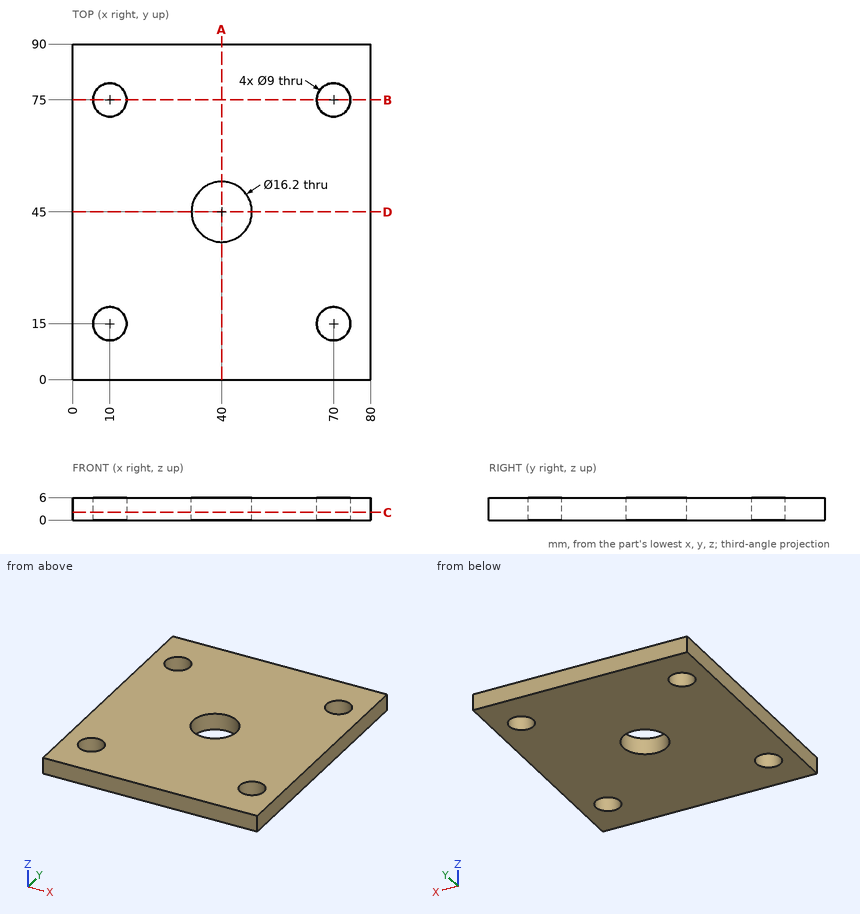
Part print with two shaded views. Sizes in mm from the minimum x, y, z corner. Round coordinates to 2 decimals unless told otherwise and drop trailing zeros. Order: outer loops, then holes, each group sorted by start corner. A loop starts at its lowest first (then second) coordinate and runs counter-clockwise, first axis right, second up. Notation, with made-up numbers: M 55,-1 L 60,-1 A27 ccw 60,15 Z; hole C 71.5,25.25 d5. An arc over 180 degrees is marked long. Use CSV: the item, a comma, the result in double quotes. Start each with the question number.
(1) Cut at D-D on y = 45. List the corners of the cut face in (x, z), then the cut area to 3 significant figures.
(2) Drill centre lines: probe 1 along X at (y, z) = (75, 3.9); probe 2 along Y at (x, z) = (8.5, 3.9); probe 3 along Y at (x, z) = (73.5, 3.6). Where is each one in solid material? Low to high.
(3) Cut at C-C on z = 2.05. List the corners of the cut face in (x, y), then the cut area to 3 significant figures.
(4) Cut at A-A on x = 40. List the corners of the cut face in (y, z), then the cut area to 3 significant figures.
(5) Flat gauge pins, fed straight in: P1, Ø14.5, axis at x = 10, y = 15, coming from the -Z side; P2, Ø7, axis at x = 10, y = 75, coming from the +Z side. Where does each tip first touch, or does it go through?
(6) Cut at B-B on y = 75. List the corners of the cut face in (x, z), then the cut area to 3 significant figures.
Findings:
1,outline,"M 0,0 L 31.9,0 L 31.9,6 L 0,6 Z; M 48.1,0 L 80,0 L 80,6 L 48.1,6 Z"
1,area,"383 mm^2"
2,probe 1,"x = 0 to 5.5, 14.5 to 65.5, 74.5 to 80"
2,probe 2,"y = 0 to 10.76, 19.24 to 70.76, 79.24 to 90"
2,probe 3,"y = 0 to 12.17, 17.83 to 72.17, 77.83 to 90"
3,outline,"M 0,0 L 80,0 L 80,90 L 0,90 Z; hole C 10,15 d9; hole C 10,75 d9; hole C 40,45 d16.2; hole C 70,15 d9; hole C 70,75 d9"
3,area,"6,740 mm^2"
4,outline,"M 0,0 L 36.9,0 L 36.9,6 L 0,6 Z; M 53.1,0 L 90,0 L 90,6 L 53.1,6 Z"
4,area,"443 mm^2"
5,P1,"stops at z = 0"
5,P2,"passes through"
6,outline,"M 0,0 L 5.5,0 L 5.5,6 L 0,6 Z; M 14.5,0 L 65.5,0 L 65.5,6 L 14.5,6 Z; M 74.5,0 L 80,0 L 80,6 L 74.5,6 Z"
6,area,"372 mm^2"
